```python
from build123d import *


with BuildPart() as part:
    # Sketch1 → Revolve1 (revolve)
    with BuildSketch(Plane.XY, mode=Mode.PRIVATE) as revolve1_sk:
        Polygon((11.46, -5), (11.46, 5), (8, 5), (8, 6), (4, 6), (4, -6), (8, -6), (8, -5), align=None)
    revolve(revolve1_sk.sketch.rotate(Axis((0, 0, 0), (0, 1, 0)), 90), axis=Axis((0, 0, 0), (0, 1, 0)))

    # Sketch2 → Revolve2 (revolve)
    with BuildSketch(Plane.XY, mode=Mode.PRIVATE) as revolve2_sk:
        with BuildLine():
            Line((8, 5), (11.46, 5))
            ThreePointArc((11.46, 5), (12.269567786, 5.128131219), (13, 5.5))
            Line((13, 5.5), (13, 6))
            Line((13, 6), (8, 6))
            Line((8, 6), (8, 5))
        make_face()
        with BuildLine():
            Line((13, -5.5), (13, -6))
            Line((13, -6), (8, -6))
            Line((8, -6), (8, -5))
            Line((8, -5), (11.46, -5))
            ThreePointArc((11.46, -5), (12.269567786, -5.128131219), (13, -5.5))
        make_face()
    revolve(revolve2_sk.sketch.rotate(Axis((0, 0, 0), (0, 1, 0)), 90), axis=Axis((0, 0, 0), (0, 1, 0)))


solid = part.part
```
Work out the finished part from the listing and answer in its coordinate system (mm). Coordinates: 2 decimals unless noted, no trailing zeros. Write each loop counter-clockwise with the first axis right and the second up, starting at its lowest first coordinate (ties: lowest second). Pieces come first, ordered by that corner, then holes.
Q1. A cutting plane is placed at B-B, the plane x = 0. Give the vertices of the cut face in (y, z), then the cut area to 3 significant figures.
Q2. A cutting plane is placed at A-A, the plane z = 0. Give the vertices of the cut face in (x, y).
Q3. Each of these flat-tipped pins is pushed along its axis until it touches: pin 1 Ø1.5 at (y, z) = (-1.5, 6.5) entering from -X; pin 2 Ø2 at (x, y) = (-0.5, -0.5) entering from -Z; pin 3 Ø6 at (x, y) = (-3, -3) entering from -Z. Where does it stop, or does it pass through?
Q4. A cutting plane is placed at C-C, the plane y = -3.25. Give the vertices of the cut face in (x, z).
Q5. Determine the mould class of faces 1 (the face through (3.905, -0.084, 0.867)), 2 (the face through (6.973, 0.07, 9.094)), 3 (the face through (-3, -6, -3)) for opening direction X: released by +X, released by -X, zero draft, split by the parting line, or undercut.
Q6. Find the intervals of material crossed by line 1 (Z direction, x = 0.25, y = 3.75); line 2 (X direction, y = 3.75, z = 0); line 3 (Z direction, x = -3, y = 1.25), in increasing order.
Findings below:
1. outline: (-6, -13) - (-5.5, -13) arc R2.62 ccw to (-5, -11.46) - (5, -11.46) arc R2.62 ccw to (5.5, -13) - (6, -13) - (6, -4) - (-6, -4) - close; (-6, 4) - (6, 4) - (6, 13) - (5.5, 13) arc R2.62 ccw to (5, 11.46) - (-5, 11.46) arc R2.62 ccw to (-5.5, 13) - (-6, 13) - close
1. area: 184 mm2
2. outline: (-13, -6) - (-4, -6) - (-4, 6) - (-13, 6) - (-13, 5.5) arc R2.62 ccw to (-11.46, 5) - (-11.46, -5) arc R2.62 ccw to (-13, -5.5) - close; (4, -6) - (13, -6) - (13, -5.5) arc R2.62 ccw to (11.46, -5) - (11.46, 5) arc R2.62 ccw to (13, 5.5) - (13, 6) - (4, 6) - close
3. pin 1: stops at x = -9.91
3. pin 2: stops at z = -11.46
3. pin 3: stops at z = -12.93
4. outline: circle Ø22.92 at (0, 0); hole circle Ø8 at (0, 0)
5. face 1: undercut
5. face 2: split by the parting line
5. face 3: zero draft
6. line 1: z = -11.46 to -3.99, 3.99 to 11.46
6. line 2: x = -11.46 to -4, 4 to 11.46
6. line 3: z = -11.06 to -2.65, 2.65 to 11.06
